Check sheet for the modelled part. Datum: model origin and axes. Units: mm. Face numbers are marked on the shaded views. A direction names the side the tool comes from. Give positions to 0.01 mm unless a question says otherwise; leave off trailing zeros. Loops run counter-clockwise (first coordinate to the right, second up) from the corner with the lowest first, then second, coordinate; pieces in that order, holes last.
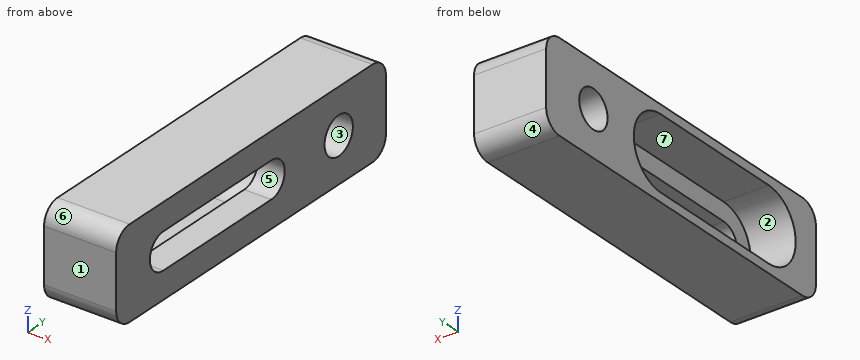
```python
from build123d import *

# Parameters (mm, degrees)
SKETCH_1_W             = 8
SKETCH_1_H             = 40
EXTRUDE_1_DEPTH        = 10
HOLE_WIZARD_M5_1_D     = 4.2
HOLE_WIZARD_M5_1_DEPTH = 12.4
HOLE_WIZARD_M5_1_TIP   = 1.2618073
FILLET_1_R             = 2
CUT_EXTRUDE_1_DEPTH    = 51.185056966
CUT_EXTRUDE_2_DEPTH    = 5
FILLET_2_R             = 2


with BuildPart() as part:
    # 草图1 → 凸台-拉伸1 (new body)
    with BuildSketch(Plane.XY):
        with Locations((-5.75595287, 28.523601913)):
            Rectangle(SKETCH_1_W, SKETCH_1_H)
    extrude(amount=EXTRUDE_1_DEPTH)

    # M5 螺纹孔1
    with Locations(Plane(origin=(-1.75595287, 0, 0), x_dir=(0, 0, -1), z_dir=(1, 0, 0))):
        with Locations((-5, 41.523601913)):
            Hole(HOLE_WIZARD_M5_1_D / 2, depth=HOLE_WIZARD_M5_1_DEPTH)
            with Locations((0, 0, -(HOLE_WIZARD_M5_1_DEPTH + HOLE_WIZARD_M5_1_TIP / 2))):  # 118° drill point
                Cone(0, HOLE_WIZARD_M5_1_D / 2, HOLE_WIZARD_M5_1_TIP, mode=Mode.SUBTRACT)

    # 圆角1
    fillet_1_edges = [part.edges().sort_by_distance(p)[0] for p in [
        (-5.75595287, 48.523601913, 10),
        (-5.75595287, 48.523601913, 0),
    ]]
    fillet(fillet_1_edges, radius=FILLET_1_R)

    # 草图5 → 切除-拉伸1 (cut, through all)
    with BuildSketch(Plane.ZY.offset(9.75595287)):
        with BuildLine():
            Line((3, 15.523601913), (3, 31.523601913))
            ThreePointArc((3, 31.523601913), (5, 33.523601913), (7, 31.523601913))
            Line((7, 31.523601913), (7, 15.523601913))
            ThreePointArc((7, 15.523601913), (5, 13.523601913), (3, 15.523601913))
        make_face()
    extrude(amount=-CUT_EXTRUDE_1_DEPTH, mode=Mode.SUBTRACT)

    # 草图6 → 切除-拉伸2 (cut)
    with BuildSketch(Plane.ZY.offset(9.75595287)):
        with BuildLine():
            Line((9, 31.523601913), (9, 15.523601913))
            ThreePointArc((9, 15.523601913), (5, 11.523601913), (1, 15.523601913))
            Line((1, 15.523601913), (1, 31.523601913))
            ThreePointArc((1, 31.523601913), (5, 35.523601913), (9, 31.523601913))
        make_face()
    extrude(amount=-CUT_EXTRUDE_2_DEPTH, mode=Mode.SUBTRACT)

    # 圆角2
    fillet_2_edges = [part.edges().sort_by_distance(p)[0] for p in [
        (-5.75595287, 8.523601913, 10),
        (-5.75595287, 8.523601913, 0),
    ]]
    fillet(fillet_2_edges, radius=FILLET_2_R)


solid = part.part
```
(1) Release check for a two-part mould opening along Y. For the marked faces 1, 2, 3 and 4 record: pulls with the +Y half, pulls with the -Y half, needs draft (parallel to the pull), parting line crosses it, or undercut.
(2) Gauge pin test, flat end, axial feed: pin 1 Ø2.5 at (y, z) = (28.5, 6.5) entering from -X. Record the tip position at first contact, or that the pin passes through.
(3) Access from +Z, -Z, +X, -X, +Y, -Y to the whole of each face (thin tool, end or side, straight path). Record for the marked faces 5, 6 and 7.
(4) Section check B-B on z = 5. Record the boundary of the cut face in (x, y), plus the area to 3 significant figures.
(5) Section check D-D on y = 43. Record the boundary of the cut face in (x, z).
(6) Material ranges on line 1 (Y direction, x = -6, z = 5); line 2 (Z direction, x = -7.5, y = 24.5); line 3 (Z direction, x = -2.5, y = 26.5), recorded low to high.
(7) Section check C-C on x = -3. Record the boundary of the cut face in (y, z).
(8) Section check A-A on y = 25. Record the boundary of the cut face in (x, z), plus the area to 3 significant figures.
Computed values:
1. face 1: pulls with the -Y half
1. face 2: undercut
1. face 3: undercut
1. face 4: pulls with the +Y half
2. pin 1: stops at x = -4.76
3. face 5: +X, -X
3. face 6: +Z, +X, -X, -Y
3. face 7: -X
4. outline: (-9.76, 8.52) - (-1.76, 8.52) - (-1.76, 13.52) - (-4.76, 13.52) - (-4.76, 11.52) - (-9.76, 11.52) - close; (-9.76, 35.52) - (-4.76, 35.52) - (-4.76, 33.52) - (-1.76, 33.52) - (-1.76, 39.42) - (-9.76, 39.42) - close; (-9.76, 43.62) - (-1.76, 43.62) - (-1.76, 48.52) - (-9.76, 48.52) - close
4. area: 106 mm2
5. outline: (-9.76, 0) - (-1.76, 0) - (-1.76, 3.51) - (-9.76, 3.51) - close; (-9.76, 6.49) - (-1.76, 6.49) - (-1.76, 10) - (-9.76, 10) - close
6. line 1: y = 8.52 to 11.52, 35.52 to 39.42, 43.62 to 48.52
6. line 2: z = 0 to 1, 9 to 10
6. line 3: z = 0 to 3, 7 to 10
7. outline: (8.52, 2) arc R2 ccw to (10.52, 0) - (46.52, 0) arc R2 ccw to (48.52, 2) - (48.52, 8) arc R2 ccw to (46.52, 10) - (10.52, 10) arc R2 ccw to (8.52, 8) - close; hole (15.52, 3) - (31.52, 3) arc R2 ccw to (31.52, 7) - (15.52, 7) arc R2 ccw to start; hole circle Ø4.2 at (41.52, 5)
8. outline: (-9.76, 0) - (-1.76, 0) - (-1.76, 3) - (-4.76, 3) - (-4.76, 1) - (-9.76, 1) - close; (-9.76, 9) - (-4.76, 9) - (-4.76, 7) - (-1.76, 7) - (-1.76, 10) - (-9.76, 10) - close
8. area: 28.0 mm2
